Check sheet for the modelled part. Datum: model origin and axes. Units: mm. Face numbers are marked on the shaded views. Round coordinates to 2 decimals unless told otherwise and drop trailing zeros. Write each loop counter-clockwise with the first axis right and the second up, starting at its lowest first coordinate (ties: lowest second). Pieces come first, ordered by that corner, then holes. Notation, with made-up numbers: (68.5, -38.75) -> (112.5, -38.75) arc R29 ccw to (112.5, -8.75) -> close; hole circle Ø10 at (-37.5, 36). An arc over 180 degrees is marked (long way). One line per item, written item: value.
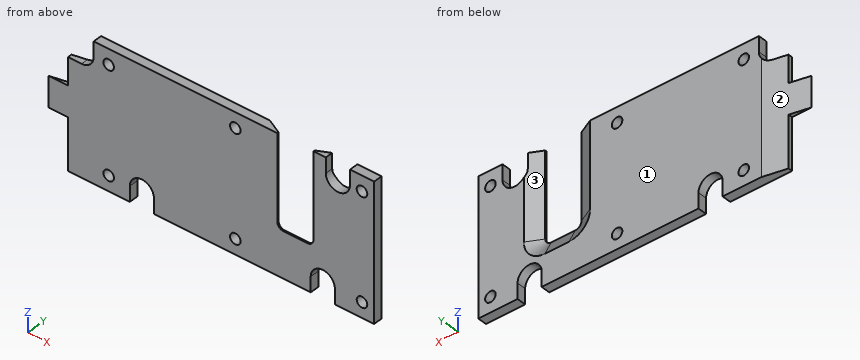
from build123d import *

# Parameters (mm, degrees)
SKETCH1_W           = 104.5
SKETCH1_H           = 45
BOSS_EXTRUDE1_DEPTH = 3
SKETCH2_W           = 12
SKETCH2_H           = 30
CUT_EXTRUDE1_DEPTH  = 34
SKETCH3_W           = 3
SKETCH3_H           = 45
CUT_EXTRUDE2_DEPTH  = 10
SKETCH4_R           = 1.75
CUT_EXTRUDE3_DEPTH  = 10
SKETCH5_W           = 10
SKETCH5_H           = 3
BOSS_EXTRUDE2_DEPTH = 6.5
CUT_EXTRUDE4_DEPTH  = 75.064583304
SKETCH7_R           = 4
CUT_EXTRUDE5_DEPTH  = 10
SKETCH8_W           = 8
SKETCH8_H           = 8.668176015
CUT_EXTRUDE6_DEPTH  = 10
FILLET1_R           = 2
CHAMFER2_SIZE       = 5
CHAMFER2_SIZE2      = 2.5


with BuildPart() as part:
    # Sketch1 → Boss-Extrude1 (new body)
    with BuildSketch(Plane(origin=(0, 0, 0), x_dir=(1, 0, 0), z_dir=(0, 1, 0))):
        Rectangle(SKETCH1_W, SKETCH1_H)
    extrude(amount=BOSS_EXTRUDE1_DEPTH)

    # Sketch2 → Cut-Extrude1 (cut)
    with BuildSketch(Plane(origin=(0, 3, 0), x_dir=(1, 0, 0), z_dir=(0, 1, 0))):
        with Locations((23.17, -7.5)):
            Rectangle(SKETCH2_W, SKETCH2_H)
    extrude(amount=-CUT_EXTRUDE1_DEPTH, mode=Mode.SUBTRACT)

    # Sketch3 → Cut-Extrude2 (cut)
    with BuildSketch(Plane(origin=(0, 3, 0), x_dir=(1, 0, 0), z_dir=(0, 1, 0))):
        with Locations((50.75, 0)):
            Rectangle(SKETCH3_W, SKETCH3_H)
    extrude(amount=-CUT_EXTRUDE2_DEPTH, mode=Mode.SUBTRACT)

    # Sketch4 → Cut-Extrude3 (cut)
    with BuildSketch(Plane(origin=(0, 3, 0), x_dir=(1, 0, 0), z_dir=(0, 1, 0))):
        with Locations(Location((45.25, 17.5, 0), (0, 0, 270))):
            Circle(SKETCH4_R)
        with Locations(Location((45.25, -17.5, 0), (0, 0, 270))):
            Circle(SKETCH4_R)
        with Locations(Location((-38.75, 17.5, 0), (0, 0, 270))):
            Circle(SKETCH4_R)
        with Locations(Location((3.25, 17.5, 0), (0, 0, 270))):
            Circle(SKETCH4_R)
        with Locations(Location((-38.75, -17.5, 0), (0, 0, 270))):
            Circle(SKETCH4_R)
        with Locations(Location((3.25, -17.5, 0), (0, 0, 270))):
            Circle(SKETCH4_R)
    extrude(amount=-CUT_EXTRUDE3_DEPTH, mode=Mode.SUBTRACT)

    # Sketch5 → Boss-Extrude2 (add)
    with BuildSketch(Plane.ZY.offset(52.25)):
        with Locations((-0.5, 1.5)):
            Rectangle(SKETCH5_W, SKETCH5_H)
    extrude(amount=BOSS_EXTRUDE2_DEPTH)

    # Sketch6 → Cut-Extrude4 (cut, through all)
    with BuildSketch(Plane.XY.offset(22.5)):
        Polygon((-58.75, 0), (-44.636109672, 3), (-58.75, 3), align=None)
    extrude(amount=-CUT_EXTRUDE4_DEPTH, mode=Mode.SUBTRACT)

    # Sketch7 → Cut-Extrude5 (cut)
    with BuildSketch(Plane(origin=(0, 3, 0), x_dir=(1, 0, 0), z_dir=(0, 1, 0))):
        with Locations(Location((-27.75, 17.5, 0), (0, 0, 270))):
            Circle(SKETCH7_R)
        with Locations(Location((-47.75, -17.5, 0), (0, 0, 270))):
            Circle(SKETCH7_R)
        with Locations(Location((32.25, 17.5, 0), (0, 0, 270))):
            Circle(SKETCH7_R)
        with Locations(Location((37.25, -17.5, 0), (0, 0, 270))):
            Circle(SKETCH7_R)
    extrude(amount=-CUT_EXTRUDE5_DEPTH, mode=Mode.SUBTRACT)

    # Sketch8 → Cut-Extrude6 (cut)
    with BuildSketch(Plane(origin=(0, 3, 0), x_dir=(1, 0, 0), z_dir=(0, 1, 0))):
        with Locations((-27.75, 21.834088008)):
            Rectangle(SKETCH8_W, SKETCH8_H)
        with Locations((32.25, 21.834088008)):
            Rectangle(SKETCH8_W, SKETCH8_H)
        with BuildLine():
            Line((41.25, -17.5), (41.25, -22.5))
            Line((41.25, -22.5), (33.25, -22.5))
            Line((33.25, -22.5), (33.25, -17.5))
            ThreePointArc((33.25, -17.5), (37.25, -13.5), (41.25, -17.5))
        make_face()
        with BuildLine():
            Line((-43.75, -17.5), (-43.75, -22.5))
            Line((-43.75, -22.5), (-52.25, -22.5))
            Line((-52.25, -22.5), (-52.25, -13.5))
            Line((-52.25, -13.5), (-47.75, -13.5))
            ThreePointArc((-47.75, -13.5), (-44.921572875, -14.671572875), (-43.75, -17.5))
        make_face()
    extrude(amount=-CUT_EXTRUDE6_DEPTH, mode=Mode.SUBTRACT)

    # Fillet1
    fillet1_edges = [part.edges().sort_by_distance(p)[0] for p in [
        (29.17, 1.5, -7.5),
        (17.17, 1.5, -7.5),
    ]]
    fillet(fillet1_edges, radius=FILLET1_R)

    # Chamfer2
    chamfer2_edges = [part.edges().sort_by_distance(p)[0] for p in [
        (29.17, 3, 8.5),
        (28.584213562, 3, -6.914213562),
        (23.17, 3, -7.5),
        (17.755786438, 3, -6.914213562),
        (17.17, 3, 8.5),
    ]]
    chamfer2_side = [part.faces().sort_by_distance(p)[0] for p in [
        (-0.332275855, 3, -0.451474159),
    ]]
    chamfer(chamfer2_edges, length=CHAMFER2_SIZE, length2=CHAMFER2_SIZE2, reference=chamfer2_side[0])


solid = part.part
Item 1: Sectioned sample at A-A (x = 3.25). Enter the section's corners in (y, z), then the cut area to 3 significant figures.
Result set:
outline: (0, -22.5) -> (3, -22.5) -> (3, -19.25) -> (0, -19.25) -> close; (0, -15.75) -> (3, -15.75) -> (3, 15.75) -> (0, 15.75) -> close; (0, 19.25) -> (3, 19.25) -> (3, 22.5) -> (0, 22.5) -> close
area: 114 mm^2
Item 2: Sectioned sample at D-D (x = 37.25). Enter the section's corners in (y, z).
Result set:
outline: (0, -22.5) -> (3, -22.5) -> (3, 13.5) -> (0, 13.5) -> close
Item 3: Sectioned sample at C-C (z = 11). Enter the section's corners in (x, y).
Result set:
outline: (-52.25, 0) -> (17.17, 0) -> (17.17, 0.5) -> (12.17, 3) -> (-44.64, 3) -> (-52.25, 1.38) -> close; (29.17, 0) -> (49.25, 0) -> (49.25, 3) -> (34.17, 3) -> (29.17, 0.5) -> close
Item 4: Depth check by flat-ended pin: pin 1 (0.7 mm diameter, centred on y = 1, z = 7.5, fed in from -X); pin 2 (3 mm diameter, centred on x = 3.25, z = -17.5, fed in from +Y); pin 3 (1.2 mm diameter, centred on x = -51, y = 1.5, fed in from +Z). Enter the tip coordinate at first touch or a pass-through.
Result set:
pin 1: x = -52.25
pin 2: through
pin 3: z = 13.5
Item 5: Sectioned sample at B-B (z = 0). Enter the section's corners in (x, y).
Result set:
outline: (-58.75, 0) -> (17.17, 0) -> (17.17, 0.5) -> (12.17, 3) -> (-44.64, 3) -> close; (29.17, 0) -> (49.25, 0) -> (49.25, 3) -> (34.17, 3) -> (29.17, 0.5) -> close
Item 6: Material ranges on line 1 along X through (y, z) = (2.25, 17.5); line 2 along X through (y, z) = (2.65, 19); line 3 along X through (y, z) = (0.9, 17.5), recorded low to high.
Result set:
line 1: -43.75 to -40.5, -37 to 1.5, 5 to 13.67, 32.67 to 33.25, 41.25 to 43.5, 47 to 49.25
line 2: -43.75 to -39.65, -37.85 to 2.35, 4.15 to 12.87, 41.25 to 44.35, 46.15 to 49.25
line 3: -43.75 to -40.5, -37 to 1.5, 5 to 16.37, 29.97 to 33.25, 41.25 to 43.5, 47 to 49.25
Item 7: Release check for a two-part mould opening along X. For the marked faces 1, 2 and 3 record: pulls with the +X half, pulls with the -X half, needs draft (parallel to the pull), parting line crosses it, or undercut.
Result set:
face 1: needs draft
face 2: pulls with the -X half
face 3: undercut
